For this review, use the dimensioned drawing (mm, ordinates from the lowest corner) and the shaded views. A direction names the side the tool comes from. Coordinates: 2 decimals unless noted, no trailing zeros. Order: outer loops, then holes, each group sorted by start corner. A loop starts at its lowest first (then second) coordinate and runs counter-clockwise, first axis right, second up. Notation, with made-up numbers: M 7.5,64.5 L 14.5,64.5 A16 ccw 14.5,87.5 Z; hole C 17.5,23.25 d7. An arc over 180 degrees is marked long. One line per item, written item: value.
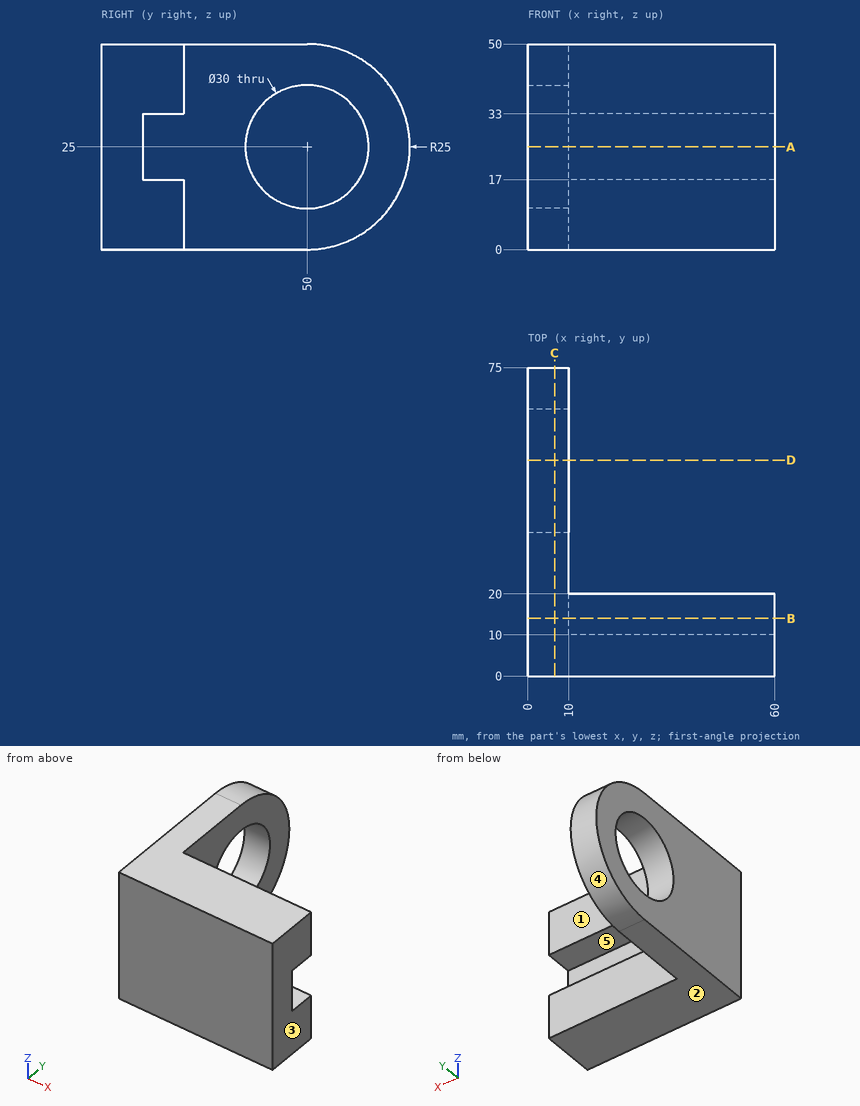
(1) We need section A-A, the plane z = 25. State the section outline as (x, y) points.
Geometry results:
outline: M 0,0 L 60,0 L 60,10 L 10,10 L 10,35 L 0,35 Z; M 0,65 L 10,65 L 10,75 L 0,75 Z
(2) We need section B-B, the plane y = 14. State the section outline as (x, z) points, plus the area to 3 significant figures.
Geometry results:
outline: M 0,0 L 60,0 L 60,17 L 10,17 L 10,33 L 60,33 L 60,50 L 0,50 Z
area: 2,200 mm2
(3) Mouldability with a two-part tool opening along Z and no side actions: class the marked faces 3, 4 and 5 as +Z half, -Z half, draft (parallel to the pull), parting line (faces both ways), or undercut.
Geometry results:
face 3: draft
face 4: parting line
face 5: undercut
(4) Insertion check: pin 1 Ø13.5 at (x, z) = (23.5, 6) entering from +Y; pin 2 Ø1 at (y, z) = (35, 17.5) entering from +X; pin 3 Ø4 at (x, z) = (40.5, 30) entering from +Y. Each pin has a flat end and moves straight along its axis. Give the tip position at first contact, or say it passes through.
Geometry results:
pin 1: stops at y = 20
pin 2: stops at x = 10
pin 3: stops at y = 10
(5) For L1, parallel to Y at x = 6.75, z = 25; L2, parallel to X at y = 32.5, z = 2, list the stretches that pass through material, from the lowest coordinate up.
Geometry results:
L1: y = 0 to 35, 65 to 75
L2: x = 0 to 10
(6) Tool access review of the marked faces 1 and 2: name each direction out of +Z, -Z, +X, -X, +Y, -Y from which nothing blocks a thin tool from reaching the whole face with its end or side.
Geometry results:
face 1: +Z, -Z, +X, +Y
face 2: -Z, +X, -X, +Y, -Y
(7) We need section C-C, the plane x = 6.5. State the section outline as (y, z) points, plus the area to 3 significant figures.
Geometry results:
outline: M 0,0 L 50,0 A25 ccw 50,50 L 0,50 Z; hole C 50,25 d30
area: 2,770 mm2
(8) We need section D-D, the plane y = 52.5. State the section outline as (x, z) points.
Geometry results:
outline: M 0,0.13 L 10,0.13 L 10,10.21 L 0,10.21 Z; M 0,39.79 L 10,39.79 L 10,49.87 L 0,49.87 Z
